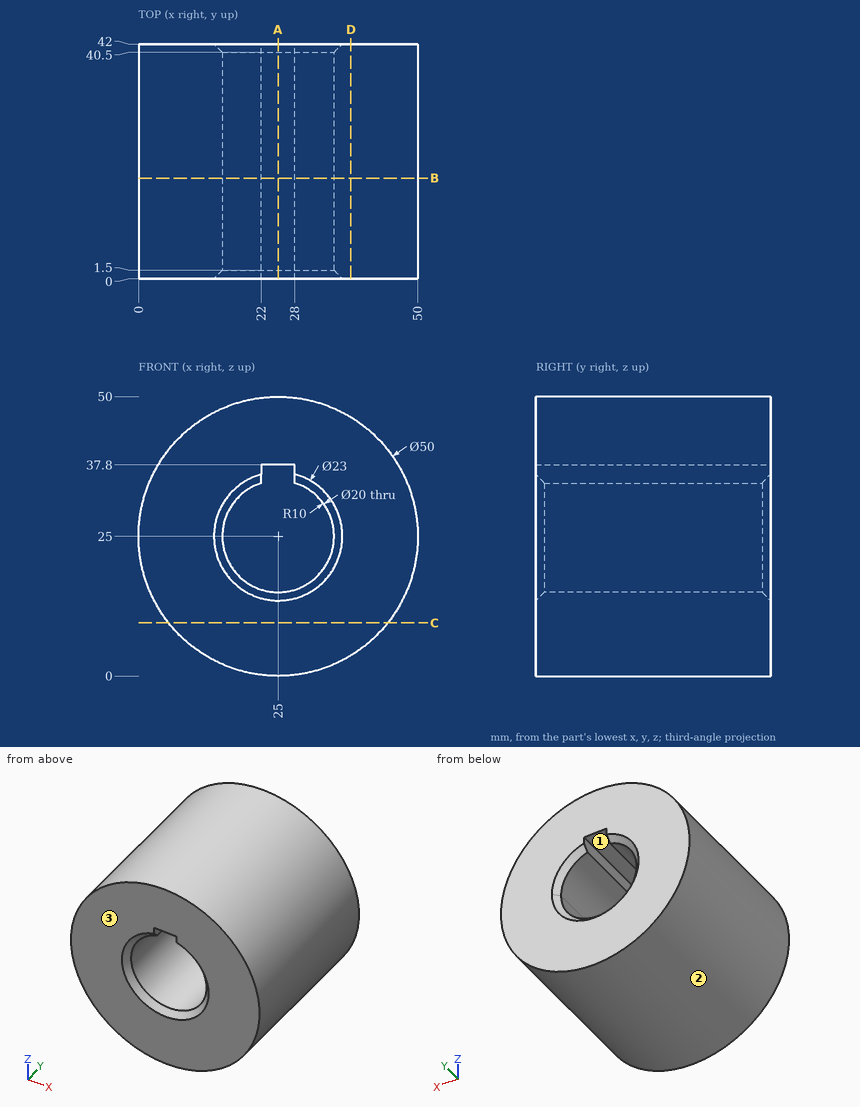
Can you work these out from the drawing? Everything is in mm from the part's minimum corner. Round coordinates to 2 decimals unless told otherwise and drop trailing zeros. Order: outer loops, then holes, each group sorted by start corner. A loop starts at its lowest first (then second) coordinate and runs counter-clockwise, first axis right, second up. Notation, with made-up numbers: (66.5, 20) - (91.5, 20) arc R19 ccw to (91.5, 46) - close; hole circle Ø9 at (44.25, 40). An arc over 180 degrees is marked (long way). Answer in a Markdown table with one row per item.
(1) Suppose I cut it at B-B, the plane y = 18. Please give me the cut outline in (x, z).
From the geometry:
| item | result |
|---|---|
| outline | circle Ø50 at (25, 25); hole (22, 34.54) arc R10 ccw (long way) to (28, 34.54) - (28, 37.8) - (22, 37.8) - close |
(2) If we mould it in two halves opening along X, with no side actions, what happens to the marked faces 1, 2 and 3? For each: released by +X, released by -X, zero draft, split by the parting line, or undercut.
From the geometry:
| item | result |
|---|---|
| face 1 | undercut |
| face 2 | split by the parting line |
| face 3 | zero draft |
(3) Suppose I cut it at C-C, the plane z = 9.5. Please give me the cut outline in (x, y).
From the geometry:
| item | result |
|---|---|
| outline | (5.38, 0) - (44.62, 0) - (44.62, 42) - (5.38, 42) - close |
(4) Suppose I cut it at A-A, the plane x = 25. Please give me the cut outline in (y, z), plus the area to 3 significant figures.
From the geometry:
| item | result |
|---|---|
| outline | (0, 0) - (42, 0) - (42, 13.5) - (40.5, 15) - (1.5, 15) - (0, 13.5) - close; (0, 37.8) - (42, 37.8) - (42, 50) - (0, 50) - close |
| area | 1,140 mm2 |
(5) Suppose I cut it at D-D, the plane x = 38. Please give me the cut outline in (y, z), plus the area to 3 significant figures.
From the geometry:
| item | result |
|---|---|
| outline | (0, 3.65) - (42, 3.65) - (42, 46.35) - (0, 46.35) - close |
| area | 1,790 mm2 |
(6) Please list where these lines run through material, in increasing order: L1, parallel to X at y = 10, z = 25; L2, parallel to X at y = 22, z = 33; L3, parallel to Z at x = 33.5, y = 23.5. Write a range as from..to.
From the geometry:
| item | result |
|---|---|
| L1 | x = 0..15, 35..50 |
| L2 | x = 1.31..19, 31..48.69 |
| L3 | z = 1.49..19.73, 30.27..48.51 |
(7) For P1, Ø12, axis at y = 30.5, z = 29, coming from the -X side; P2, Ø8, axis at y = 30, z = 34, coming from the +X side; P3, Ø3.5, axis at y = 12, z = 36, coming from the -X side, each with a flat end and sliding along its axis, tell me the tip position at first contact or that it passes through.
From the geometry:
| item | result |
|---|---|
| P1 | stops at x = 0 |
| P2 | stops at x = 49.49 |
| P3 | stops at x = 1.77 |
